from build123d import *

# Parameters (mm, degrees)
SKETCH_1_R      = 6
EXTRUDE_1_DEPTH = 3.74
SKETCH_2_R      = 4
EXTRUDE_2_DEPTH = 5
SKETCH_3_R      = 3
EXTRUDE_3_DEPTH = 8


with BuildPart() as part:
    # 草图1 → 凸台-拉伸1 (new body)
    with BuildSketch(Plane.XY):
        Circle(SKETCH_1_R)
    extrude(amount=EXTRUDE_1_DEPTH)

    # 草图2 → 凸台-拉伸2 (add)
    with BuildSketch(Plane.XY.offset(3.74)):
        Circle(SKETCH_2_R)
    extrude(amount=EXTRUDE_2_DEPTH)

    # 草图3 → 凸台-拉伸3 (add)
    with BuildSketch(Plane.XY.offset(8.74)):
        Circle(SKETCH_3_R)
    extrude(amount=EXTRUDE_3_DEPTH)


solid = part.part
Can you work these out from the model? Positions are in its coordinate system, mm. A direction names the side the tool comes from. Give positions to 0.01 mm unless a question says otherwise; leave off trailing zeros. Loops run counter-clockwise (first coordinate to the right, second up) from the corner with the lowest first, then second, coordinate; pieces in that order, holes last. Notation, with made-up numbers: (65.5, -35.5) -> (72.5, -35.5) arc R17 ccw to (72.5, -28.5) -> close; hole circle Ø3 at (-25, -16). An arc over 180 degrees is marked (long way). Return JSON: item names as keys, results as strings.
Q1. I want a section at A-A, the plane x = 0. List the corners of the cut face in (y, z) for me.
Checks:
{"outline": "(-6, 0) -> (6, 0) -> (6, 3.74) -> (4, 3.74) -> (4, 8.74) -> (3, 8.74) -> (3, 16.74) -> (-3, 16.74) -> (-3, 8.74) -> (-4, 8.74) -> (-4, 3.74) -> (-6, 3.74) -> close"}
Q2. On a 3-axis mill with a long thin cutter (end or side, diameter ignored), from which of +Z, -Z, +X, -X, +Y, -Y can I reach the whole of each face in a straight line? I mean faces 1 (the face through (1, 3, 8.74)), 2 (the face through (0, 0, 16.74)). Say none if no direction works.
Checks:
{"face 1": "+Z", "face 2": "+Z, +X, -X, +Y, -Y"}
Q3. For pin 1 Ø3 at (x, z) = (4, 6.5) entering from -Y; pin 2 Ø6 at (y, z) = (-4, 5) entering from -X; pin 3 Ø4 at (x, z) = (-1.5, 9) entering from -Y, each with a flat end and sliding along its axis, tell me the tip position at first contact or that it passes through.
Checks:
{"pin 1": "stops at y = -3.12", "pin 2": "stops at x = -5.86", "pin 3": "stops at y = -4"}
Q4. I want a section at D-D, the plane z = 9.5. List the corners of the cut face in (x, y) for me, then the cut area to 3 significant figures.
Checks:
{"outline": "circle Ø6 at (0, 0)", "area": "28.3 mm2"}
Q5. I need wall thicknesses on probe 1 along Z at (x, y) = (-2.25, 4); probe 2 along Y at (x, z) = (0.75, 1.25); probe 3 along Y at (x, z) = (-1, 8.5). Which ranges of each line are inside material? Lowest first, please.
Checks:
{"probe 1": "z = 0 to 3.74", "probe 2": "y = -5.95 to 5.95", "probe 3": "y = -3.87 to 3.87"}
Q6. I want a section at C-C, the plane z = 3. List the corners of the cut face in (x, y) for me, then the cut area to 3 significant figures.
Checks:
{"outline": "circle Ø12 at (0, 0)", "area": "113 mm2"}
